from build123d import *

# Parameters (mm, degrees)
FLANGE_DISC_SKETCH_300_R         = 150
FLANGE_DISC_300X40_DEPTH         = 40
BORE_SKETCH_70_R                 = 35
BORE_70_THROUGH_DEPTH            = 40
BORE_RECESS_SKETCH_80_3_R        = 40.15
BORE_RECESS_SKETCH_80_3_R_2      = 35
BORE_RECESS_80_3X5_DEPTH         = 5
RAISED_FACE_STEP_SKETCH_R        = 150
RAISED_FACE_STEP_SKETCH_R_2      = 97.5
RAISED_FACE_STEP_195X10_DEPTH    = 10
OUTER_BOLT_HOLES_SKETCH_PCD254_R = 11.75
OUTER_BOLT_HOLES_PCD254_DEPTH    = 215.242852856
INNER_HOLES_SKETCH_R             = 17.5
INNER_HOLES_CUT_24_DEEP_DEPTH    = 24
INNER_HOLE_SECONDARY_SKETCH_R    = 11.5
INNER_HOLE_SECONDARY_CUT_DEPTH   = 216.870331449
SMALL_HOLE_SKETCH_12_R           = 6
SMALL_HOLE_12_DEPTH              = 216.870331449


with BuildPart() as part:
    # Flange Disc Sketch Ø300 → Flange Disc Ø300x40 (new body)
    with BuildSketch(Plane(origin=(0, 0, 0), x_dir=(1, 0, 0), z_dir=(0, 1, 0))):
        with Locations(Location((0, 0, 0), (0, 0, 270))):
            Circle(FLANGE_DISC_SKETCH_300_R)
    extrude(amount=-FLANGE_DISC_300X40_DEPTH)

    # Bore Sketch Ø70 → Bore Ø70 Through (cut)
    with BuildSketch(Plane(origin=(0, 0, 0), x_dir=(1, 0, 0), z_dir=(0, 1, 0))):
        with Locations(Location((0, 0, 0), (0, 0, 270))):
            Circle(BORE_SKETCH_70_R)
    extrude(amount=-BORE_70_THROUGH_DEPTH, mode=Mode.SUBTRACT)

    # Bore Recess Sketch Ø80.3 → Bore Recess Ø80.3x5 (cut)
    with BuildSketch(Plane(origin=(0, 0, 0), x_dir=(1, 0, 0), z_dir=(0, 1, 0))):
        with Locations(Location((0, 0, 0), (0, 0, 270))):
            Circle(BORE_RECESS_SKETCH_80_3_R)
        with Locations(Location((0, 0, 0), (0, 0, 270))):
            Circle(BORE_RECESS_SKETCH_80_3_R_2, mode=Mode.SUBTRACT)
    extrude(amount=-BORE_RECESS_80_3X5_DEPTH, mode=Mode.SUBTRACT)

    # Raised Face Step Sketch → Raised Face Step Ø195x10 (cut)
    with BuildSketch(Plane(origin=(0, 0, 0), x_dir=(1, 0, 0), z_dir=(0, 1, 0))):
        with Locations(Location((0, 0, 0), (0, 0, 270))):
            Circle(RAISED_FACE_STEP_SKETCH_R)
        with Locations(Location((0, 0, 0), (0, 0, 270))):
            Circle(RAISED_FACE_STEP_SKETCH_R_2, mode=Mode.SUBTRACT)
    extrude(amount=-RAISED_FACE_STEP_195X10_DEPTH, mode=Mode.SUBTRACT)

    # Outer Bolt Holes Sketch PCD254 → Outer Bolt Holes PCD254 (cut, through all)
    with BuildSketch(Plane(origin=(0, -10, 0), x_dir=(1, 0, 0), z_dir=(0, 1, 0))):
        with Locations(Location((89.802561211, 89.802561211, 0), (0, 0, 270))):
            Circle(OUTER_BOLT_HOLES_SKETCH_PCD254_R)
        with Locations(Location((-89.802561211, 89.802561211, 0), (0, 0, 90))):
            Circle(OUTER_BOLT_HOLES_SKETCH_PCD254_R)
        with Locations(Location((-89.802561211, -89.802561211, 0), (0, 0, 270))):
            Circle(OUTER_BOLT_HOLES_SKETCH_PCD254_R)
        with Locations(Location((89.802561211, -89.802561211, 0), (0, 0, 90))):
            Circle(OUTER_BOLT_HOLES_SKETCH_PCD254_R)
    extrude(amount=-OUTER_BOLT_HOLES_PCD254_DEPTH, mode=Mode.SUBTRACT)

    # Inner Holes Sketch → Inner Holes Cut 24 Deep (cut)
    with BuildSketch(Plane(origin=(0, 0, 0), x_dir=(1, 0, 0), z_dir=(0, 1, 0))):
        with Locations(Location((-70.476946559, -25.651510749, 0), (0, 0, 270))):
            Circle(INNER_HOLES_SKETCH_R)
        with Locations(Location((70.476946559, 25.651510749, 0), (0, 0, 270))):
            Circle(INNER_HOLES_SKETCH_R)
        with Locations(Location((-25.616759959, 70.489585112, 0), (0, 0, 270))):
            Circle(INNER_HOLES_SKETCH_R)
        with Locations(Location((25.686255305, -70.464290874, 0), (0, 0, 270))):
            Circle(INNER_HOLES_SKETCH_R)
    extrude(amount=-INNER_HOLES_CUT_24_DEEP_DEPTH, mode=Mode.SUBTRACT)

    # Inner Hole Secondary Sketch → Inner Hole Secondary Cut (cut, through all)
    with BuildSketch(Plane(origin=(0, 0, 0), x_dir=(1, 0, 0), z_dir=(0, 1, 0))):
        with Locations(Location((70.476946559, 25.651510749, 0), (0, 0, 270))):
            Circle(INNER_HOLE_SECONDARY_SKETCH_R)
        with Locations(Location((-70.407451213, -25.626216512, 0), (0, 0, 270))):
            Circle(INNER_HOLE_SECONDARY_SKETCH_R)
        with Locations(Location((-25.616759959, 70.489585112, 0), (0, 0, 270))):
            Circle(INNER_HOLE_SECONDARY_SKETCH_R)
        with Locations(Location((25.686255305, -70.464290874, 0), (0, 0, 270))):
            Circle(INNER_HOLE_SECONDARY_SKETCH_R)
    extrude(amount=-INNER_HOLE_SECONDARY_CUT_DEPTH, mode=Mode.SUBTRACT)

    # Small Hole Sketch Ø12 → Small Hole Ø12 (cut, through all)
    with BuildSketch(Plane(origin=(0, 0, 0), x_dir=(1, 0, 0), z_dir=(0, 1, 0))):
        with Locations(Location((-60, 60, 0), (0, 0, 270))):
            Circle(SMALL_HOLE_SKETCH_12_R)
    extrude(amount=-SMALL_HOLE_12_DEPTH, mode=Mode.SUBTRACT)


solid = part.part
Verification items for the finished model (mm, model axes). A direction names the side the tool comes from. Coordinates: 2 decimals unless noted, no trailing zeros. Order: outer loops, then holes, each group sorted by start corner. A loop starts at its lowest first (then second) coordinate and runs counter-clockwise, first axis right, second up. Notation, with made-up numbers: M 72.25,30 L 129.25,30 A18 cw 129.25,57 Z; hole C 73,-33 d4. An arc over 180 degrees is marked long. Write each question's results on one line, items separated by ' | '.
1) Release check for a two-part mould opening along Z. For faces 3 (the face through (12.06, -2.465, 38.296)), 4 (the face through (-86.5, -4.93, 44.99)), 5 (the face through (1, 0, 42)) record: pulls with the +Z half, pulls with the -Z half, needs draft (parallel to the pull), parting line crosses it, or undercut.
Solved:
face 3: undercut | face 4: parting line crosses it | face 5: needs draft
2) Section check A-A on x = 0. Record the cut outline in (y, z).
Solved:
outline: M -40,-150 L -10,-150 L -10,-97.5 L 0,-97.5 L 0,-40.15 L -5,-40.15 L -5,-35 L -40,-35 Z; M -40,35 L -5,35 L -5,40.15 L 0,40.15 L 0,97.5 L -10,97.5 L -10,150 L -40,150 Z
3) Section check B-B on z = 0. Record the cut outline in (x, y).
Solved:
outline: M -150,-40 L -35,-40 L -35,-5 L -40.15,-5 L -40.15,0 L -97.5,0 L -97.5,-10 L -150,-10 Z; M 35,-40 L 150,-40 L 150,-10 L 97.5,-10 L 97.5,0 L 40.15,0 L 40.15,-5 L 35,-5 Z
4) Access from +Z, -Z, +X, -X, +Y, -Y to the whole of each face (thin tool, end or side, straight path). Record for faces 1 (the face through (-87.56, -11.83, 21.86)), 2 (the face through (-32.61, -31.89, -79.62)).
Solved:
face 1: +Y | face 2: +Y, -Y
5) Gauge pin test, flat ends, axial feed: pin 1 Ø10.5 at (x, z) = (-28, -72.5) entering from +Y; pin 2 Ø6 at (x, y) = (-13, -16) entering from +Z; pin 3 Ø1.5 at (x, y) = (-5, -13.5) entering from +Z; pin 4 Ø3 at (y, z) = (-5, 26.5) entering from -X. Record the tip position at first contact, or that the pin passes through.
Solved:
pin 1: passes through | pin 2: stops at z = 149.67 | pin 3: stops at z = 149.94 | pin 4: stops at x = -94.24
6) Section check C-C on y = -33. Give the number of separate pieces and of enclosed holes in the cut face, plus the area to 3 significant figures.
Solved:
separate pieces: 1 | enclosed holes: 10 | area: 63,300 mm²
7) Scan lines: line 1 along X through (y, z) = (-32, -90.5); line 2 along Z through (x, y) = (-99, -14); line 3 along Y through (x, z) = (-21.5, 125). Record each from-to range of solid material in increasing order. Write a range as [from, to].
Solved:
line 1: x = [-119.62, -101.53], [-78.07, 78.07], [101.53, 119.62] | line 2: z = [-112.69, -97.11], [-82.49, 82.49], [97.11, 112.69] | line 3: y = [-40, -10]
